```python
from build123d import *

# Parameters (mm, degrees)
SKETCH1_W                                            = 146
SKETCH1_H                                            = 34
BOSS_EXTRUDE1_DEPTH                                  = 6
HOLE_SIZE_PER_SOCKET_HEAD_CAP_SCREW_TYPE_D           = 5.5
HOLE_SIZE_PER_SOCKET_HEAD_CAP_SCREW_TYPE_CBORE_D     = 10
HOLE_SIZE_PER_SOCKET_HEAD_CAP_SCREW_TYPE_CBORE_DEPTH = 6
M4_TAPPED_HOLE2_D                                    = 3.3
M4_TAPPED_HOLE2_DEPTH                                = 10.1
M4_TAPPED_HOLE2_TIP                                  = 0.991420021
CHAMFER1_SIZE                                        = 3
SKETCH8_W                                            = 116
SKETCH8_H                                            = 2
CUT_EXTRUDE1_DEPTH                                   = 76.907838857
M4_TAPPED_HOLE3_AT_2_COUNT                           = 2
M4_TAPPED_HOLE3_AT_2_PITCH                           = 80
SKETCH11_W                                           = 6
SKETCH11_H                                           = 30
BOSS_EXTRUDE2_DEPTH                                  = 6
CUT_EXTRUDE2_DEPTH                                   = 82.418671077
CUT_EXTRUDE3_DEPTH                                   = 82.418671077
CHAMFER2_SIZE                                        = 1


with BuildPart() as part:
    # Sketch1 → Boss-Extrude1 (new, symmetric)
    with BuildSketch(Plane(origin=(0, 0, 0), x_dir=(1, 0, 0), z_dir=(0, 1, 0))):
        Rectangle(SKETCH1_W, SKETCH1_H)
    extrude(amount=BOSS_EXTRUDE1_DEPTH, both=True)

    # Hole size per socket head cap screw type1 (through all)
    with Locations(Plane(origin=(0, 6, 0), x_dir=(1, 0, 0), z_dir=(0, 1, 0))):
        with Locations((-58, 0), (-13, 0)):
            CounterBoreHole(HOLE_SIZE_PER_SOCKET_HEAD_CAP_SCREW_TYPE_D / 2, HOLE_SIZE_PER_SOCKET_HEAD_CAP_SCREW_TYPE_CBORE_D / 2, HOLE_SIZE_PER_SOCKET_HEAD_CAP_SCREW_TYPE_CBORE_DEPTH)

    # M4 Tapped Hole2
    with Locations(Plane(origin=(73, 0, 0), x_dir=(0, 0, -1), z_dir=(1, 0, 0))):
        with Locations((-10, -1.5), (10, -1.5)):
            Hole(M4_TAPPED_HOLE2_D / 2, depth=M4_TAPPED_HOLE2_DEPTH)
            with Locations((0, 0, -(M4_TAPPED_HOLE2_DEPTH + M4_TAPPED_HOLE2_TIP / 2))):  # 118° drill point
                Cone(0, M4_TAPPED_HOLE2_D / 2, M4_TAPPED_HOLE2_TIP, mode=Mode.SUBTRACT)

    # Chamfer1
    chamfer1_edges = [part.edges().sort_by_distance(p)[0] for p in [
        (-73, 0, 17),
        (-73, 0, -17),
    ]]
    chamfer(chamfer1_edges, length=CHAMFER1_SIZE)

    # Sketch8 → Cut-Extrude1 (cut, through all)
    with BuildSketch(Plane(origin=(0, 6, 0), x_dir=(1, 0, 0), z_dir=(0, 1, 0))):
        with Locations((15, -16)):
            Rectangle(SKETCH8_W, SKETCH8_H)
        with Locations((15, 16)):
            Rectangle(SKETCH8_W, SKETCH8_H)
    extrude(amount=-CUT_EXTRUDE1_DEPTH, mode=Mode.SUBTRACT)

    # Sketch9 → M4 Tapped Hole3 (revolve, cut)
    with BuildSketch(Plane(origin=(-23, -1.5, 15), x_dir=(0, -1, 0), z_dir=(1, 0, 0))):
        Polygon((0, 0), (0, 11.091420021), (1.65, 10.1), (1.65, 0), align=None)
    m4_tapped_hole3 = revolve(axis=Axis((-23, -1.5, 21.35), (0, 0, -1)), mode=Mode.SUBTRACT)

    # M4 Tapped Hole3 at 2: M4 Tapped Hole3 ×2
    with Locations(*[(i * M4_TAPPED_HOLE3_AT_2_PITCH, 0, 0) for i in range(1, M4_TAPPED_HOLE3_AT_2_COUNT)]):
        add(m4_tapped_hole3, mode=Mode.SUBTRACT)

    # Mirror1: M4 Tapped Hole3 across plane
    add(m4_tapped_hole3.mirror(Plane.XY), mode=Mode.SUBTRACT)

    # Mirror1 copy 1 sketch → Mirror1 copy 1 (revolve, cut)
    with BuildSketch(Plane(origin=(57, -1.5, -15), x_dir=(0, -1, 0), z_dir=(1, 0, 0))):
        Polygon((0, 0), (0, -11.091420021), (1.65, -10.1), (1.65, 0), align=None)
    revolve(axis=Axis((57, -1.5, -21.35), (0, 0, -1)), mode=Mode.SUBTRACT)

    # Sketch11 → Boss-Extrude2 (add)
    with BuildSketch(Plane(origin=(0, 6, 0), x_dir=(1, 0, 0), z_dir=(0, 1, 0))):
        with Locations((70, 0)):
            Rectangle(SKETCH11_W, SKETCH11_H)
    extrude(amount=BOSS_EXTRUDE2_DEPTH)

    # Sketch12 → Cut-Extrude2 (cut, through all)
    with BuildSketch(Plane.XY.offset(17)):
        Polygon((67, 6), (-43, 6), (67, 1.19729628), align=None)
    extrude(amount=-CUT_EXTRUDE2_DEPTH, mode=Mode.SUBTRACT)

    # Sketch13 → Cut-Extrude3 (cut, through all)
    with BuildSketch(Plane.XY.offset(17)):
        Polygon((67, 12), (67, 1.19729628), (67.47165623, 12), align=None)
    extrude(amount=-CUT_EXTRUDE3_DEPTH, mode=Mode.SUBTRACT)

    # Chamfer2
    chamfer2_edges = [part.edges().sort_by_distance(p)[0] for p in [
        (57, 0.15, 15),
        (-23, 0.15, 15),
        (57, 0.15, -15),
        (-23, 0.15, -15),
    ]]
    chamfer(chamfer2_edges, length=CHAMFER2_SIZE)


solid = part.part
```
Geometry check sheet. Reference: the model listing, model coordinates, mm. A direction names the side the tool comes from. Round coordinates to 2 decimals unless told otherwise and drop trailing zeros. Write each loop counter-clockwise with the first axis right and the second up, starting at its lowest first coordinate (ties: lowest second). Pieces come first, ordered by that corner, then holes. Notation, with made-up numbers: (13, 18.25) -> (22, 18.25) arc R34 ccw to (22, 49.25) -> close; hole circle Ø11 at (-10.5, 1.25). An arc over 180 degrees is marked (long way). Put each result on its own line as item: value.
1) Cross-section at C-C, the plane x = -13. Enter the section's corners in (y, z), plus the area to 3 significant figures.
Recorded:
outline: (-6, -15) -> (4.69, -15) -> (4.69, -5) -> (0, -5) -> (0, -2.75) -> (-6, -2.75) -> close; (-6, 2.75) -> (0, 2.75) -> (0, 5) -> (4.69, 5) -> (4.69, 15) -> (-6, 15) -> close
area: 241 mm2
2) Cross-section at A-A, the plane x = -58. Enter the section's corners in (y, z), plus the area to 3 significant figures.
Recorded:
outline: (-6, -17) -> (6, -17) -> (6, -5) -> (0, -5) -> (0, -2.75) -> (-6, -2.75) -> close; (-6, 2.75) -> (0, 2.75) -> (0, 5) -> (6, 5) -> (6, 17) -> (-6, 17) -> close
area: 315 mm2
3) Access from +Z, -Z, +X, -X, +Y, -Y to the whole of each face (thin tool, end or side, straight path). Record for faces 1 (the face through (-23.28, -1.46, 4.08)), 2 (the face through (-63, 3, 0)), 3 (the face through (-71, 0, 16)), 4 (the face through (14, -1, 15)), 5 (the face through (-24.636, -1.285, -9.514)).
Recorded:
face 1: +Z
face 2: +Y
face 3: +Z, -X, +Y, -Y
face 4: +Z, +X, +Y, -Y
face 5: -Z
4) Cross-section at D-D, the plane y = 10. Enter the section's corners in (x, z), plus the area to 3 significant figures.
Recorded:
outline: (67.38, -15) -> (73, -15) -> (73, 15) -> (67.38, 15) -> close
area: 168 mm2
5) Depth check by flat-ended pin: P1, Ø5.5, axis at x = 57, y = -1.5, coming from the +Z side; P2, Ø8, axis at x = 57.5, z = -3, coming from the +Y side; P3, Ø4, axis at x = 57, y = -1.5, coming from the +Z side; P4, Ø5, axis at x = -13, z = 0, coming from the -Y side. Enter the tip coordinate at first touch or a pass-through.
Recorded:
P1: stops at z = 15
P2: stops at y = 1.79
P3: stops at z = 14.35
P4: passes through
6) Thickness scan on probe 1 along Z at (x, y) = (65, -1.5); probe 2 along Z at (x, y) = (-13, 2.7); probe 3 along X at (y, z) = (0, 5.5). Record the ranges inside material, lowest first. Write a range as from..to.
Recorded:
probe 1: z = -15..-11.65, -8.35..8.35, 11.65..15
probe 2: z = -15..-5, 5..15
probe 3: x = -73..-23.69, -22.31..56.31, 57.69..73
7) Release check for a two-part mould opening along Z. For faces 6 (the face through (67.879, -2.132, -8.476)), 7 (the face through (67.233, 6.523, 0.21)), 8 (the face through (-57, 0, 17)), 9 (the face through (62.1, -1.6, 9.7)) record: pulls with the +Z half, pulls with the -Z half, needs draft (parallel to the pull), parting line crosses it, or undercut.
Recorded:
face 6: undercut
face 7: needs draft
face 8: pulls with the +Z half
face 9: undercut
8) Cross-section at B-B, the plane z = -7. Enter the section's corners in (x, y), plus the area to 3 significant figures.
Recorded:
outline: (-73, -6) -> (73, -6) -> (73, 12) -> (67.47, 12) -> (67, 1.2) -> (-43, 6) -> (-73, 6) -> close; hole circle Ø3.3 at (-23, -1.5); hole circle Ø3.3 at (57, -1.5)
area: 1,500 mm2
